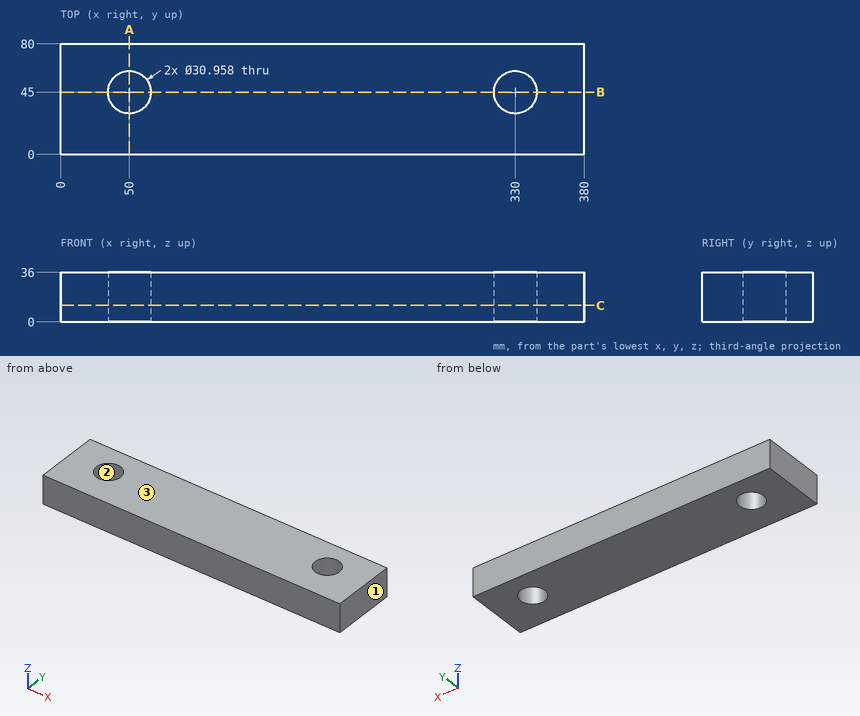
Input: dimensioned drawing with shaded views. Units: mm. Origin: part minimum x, y, z. Coordinates: 2 decimals unless noted, no trailing zeros. Write each loop counter-clockwise with the first axis right and the second up, starting at its lowest first coordinate (ties: lowest second). Pieces come first, ordered by that corner, then holes. Notation, with made-up numbers: M -35,53.5 L 8,53.5 A27 ccw 8,87.5 Z; hole C -8.75,-36 d11. An arc over 180 degrees is marked long. Answer as a JSON object with one key per item and string values. Group by question number.
(1) Section C-C on z = 12. Output: boundary loops of the cut face in (x, y), plus the area to 3 significant figures.
(2) Section A-A on x = 50. Output: boundary loops of the cut face in (y, z).
(3) Contact query for a flat-ended pin moving along its axis: P1, Ø2, axis at x = 313.5, y = 30.5, coming from the -Z side. Output: stop coordinate, or through.
(4) Mould query, pull axis X, two halves, no side actions, for the marked faces 1, 2 and 3. Classes: pulls with the +X half, pulls with the -X half, needs draft (parallel to the pull), parting line crosses it, or undercut.
(5) Section B-B on y = 45. Output: boundary loops of the cut face in (x, z).
(6) Ray query, line 1 along Y through (x, z) = (50, 19); line 2 along X through (y, z) = (42, 11.5) (1 decimal); line 3 along X through (y, z) = (56.5, 28). Return the intervals inside material, ascending. Write a range as [from, to].
Result set:
{
 "1": {"outline": "M 0,0 L 380,0 L 380,80 L 0,80 Z; hole C 50,45 d30.96; hole C 330,45 d30.96", "area": "28,900 mm2"},
 "2": {"outline": "M 0,0 L 29.52,0 L 29.52,36 L 0,36 Z; M 60.48,0 L 80,0 L 80,36 L 60.48,36 Z"},
 "3": {"P1": "stops at z = 0"},
 "4": {"face 1": "pulls with the +X half", "face 2": "undercut", "face 3": "needs draft"},
 "5": {"outline": "M 0,0 L 34.52,0 L 34.52,36 L 0,36 Z; M 65.48,0 L 314.52,0 L 314.52,36 L 65.48,36 Z; M 345.48,0 L 380,0 L 380,36 L 345.48,36 Z"},
 "6": {"line 1": "y = [0, 29.52], [60.48, 80]", "line 2": "x = [0, 34.8], [65.2, 314.8], [345.2, 380]", "line 3": "x = [0, 39.64], [60.36, 319.64], [340.36, 380]"}
}
